Read the model definition and answer for the solid it produces. Units are mm, in the model's axes. Round coordinates to 2 decimals unless told otherwise and drop trailing zeros. Write each loop counter-clockwise with the first axis right and the second up, starting at its lowest first coordinate (ties: lowest second). Pieces come first, ordered by that corner, then holes. Notation, with made-up numbers: (54.25, 65.5) - (68.25, 65.5) arc R28 cw to (68.25, 88.5) - close; hole circle Ø6 at (53, -6). An arc over 180 degrees is marked (long way). One line per item, written item: value. Start each with the question number.
(1) A cutting plane is placed at B-B, the plane x = 0. Determine the outline of the cut face in (y, z), plus the area to 3 significant figures.
(2) The mould has two halves that part along Z. Classify faces 1 (the face through (-39.706, 2.535, -26.086)), 2 (the face through (1, 5, -43)), 3 (the face through (0.811, 2.465, -62.495)): +Z half, -Z half, draft (parallel to the pull), parting line (faces both ways), or undercut.
(3) Find the intervals of material crossed by L1, parallel to X at y = 2.8, z = 25.5; L2, parallel to X at y = 0.35, z = -29.5; L3, parallel to Z at x = 45, y = 4.2, in increasing order.
(4) A cutting plane is placed at A-A, the plane z = 0. Determine the outline of the cut face in (x, y), plus the area to 3 significant figures.
(5) Flat-ended cylindrical pins translate along their axes: pin 1 Ø5.5 at (x, z) = (-44.17, -25.5) entering from +Y; pin 2 Ø3 at (x, y) = (-12.5, 3.5) entering from +Z; pin 3 Ø3 at (x, y) = (26, 4) entering from -Z; pin 4 Ø1 at (y, z) = (3.5, 48.5) entering from +X. Find the tip coordinate at first contact, or state that the pin passes through.
(6) A cutting plane is placed at C-C, the plane z = -25.5. Determine the outline of the cut face in (x, y), plus the area to 3 significant figures.
(7) A cutting plane is placed at D-D, the plane x = -37.5. Determine the outline of the cut face in (y, z), plus the area to 3 significant figures.
from build123d import *

# Parameters (mm, degrees)
SKETCH1_R           = 62.5
SKETCH1_R_2         = 42.5
BOSS_EXTRUDE1_DEPTH = 5
SKETCH2_R           = 4.5
CUT_EXTRUDE1_DEPTH  = 10
SKETCH3_OUTSIDE_W   = 162.37
SKETCH3_OUTSIDE_H   = 162.37
SKETCH3_OUTSIDE_W_2 = 100
SKETCH3_OUTSIDE_H_2 = 143.531180288
CUT_EXTRUDE2_DEPTH  = 10


with BuildPart() as part:
    # Sketch1 → Boss-Extrude1 (new body)
    with BuildSketch(Plane(origin=(0, 0, 0), x_dir=(1, 0, 0), z_dir=(0, 1, 0))):
        with Locations(Location((0, 0, 0), (0, 0, 270))):
            Circle(SKETCH1_R)
        with Locations(Location((0, 0, 0), (0, 0, 270))):
            Circle(SKETCH1_R_2, mode=Mode.SUBTRACT)
    extrude(amount=BOSS_EXTRUDE1_DEPTH)

    # Sketch2 → Cut-Extrude1 (cut)
    with BuildSketch(Plane(origin=(0, 5, 0), x_dir=(1, 0, 0), z_dir=(0, 1, 0))):
        with Locations(Location((0, 51, 0), (0, 0, 270))):
            Circle(SKETCH2_R)
        with Locations(Location((44.167295593, 25.5, 0), (0, 0, 270))):
            Circle(SKETCH2_R)
        with Locations(Location((44.167295593, -25.5, 0), (0, 0, 270))):
            Circle(SKETCH2_R)
        with Locations(Location((0, -51, 0), (0, 0, 270))):
            Circle(SKETCH2_R)
        with Locations(Location((-44.167295593, -25.5, 0), (0, 0, 270))):
            Circle(SKETCH2_R)
        with Locations(Location((-44.167295593, 25.5, 0), (0, 0, 270))):
            Circle(SKETCH2_R)
    extrude(amount=-CUT_EXTRUDE1_DEPTH, mode=Mode.SUBTRACT)

    # Sketch3 outside → Cut-Extrude2 (cut)
    with BuildSketch(Plane(origin=(0, 5, 0), x_dir=(1, 0, 0), z_dir=(0, 1, 0))):
        Rectangle(SKETCH3_OUTSIDE_W, SKETCH3_OUTSIDE_H)
        Rectangle(SKETCH3_OUTSIDE_W_2, SKETCH3_OUTSIDE_H_2, mode=Mode.SUBTRACT)
    extrude(amount=-CUT_EXTRUDE2_DEPTH, mode=Mode.SUBTRACT)


solid = part.part
Here are the results:
1. outline: (0, -62.5) - (5, -62.5) - (5, -55.5) - (0, -55.5) - close; (0, -46.5) - (5, -46.5) - (5, -42.5) - (0, -42.5) - close; (0, 42.5) - (5, 42.5) - (5, 46.5) - (0, 46.5) - close; (0, 55.5) - (5, 55.5) - (5, 62.5) - (0, 62.5) - close
1. area: 110 mm²
2. face 1: undercut
2. face 2: draft
2. face 3: -Z half
3. L1: -50 to -48.67, -39.67 to -34, 34 to 39.67, 48.67 to 50
3. L2: -50 to -46.23, -42.11 to -30.59, 30.59 to 42.11, 46.23 to 50
3. L3: -43.37 to -29.92, -21.08 to 21.08, 29.92 to 43.37
4. outline: (-50, 0) - (-42.5, 0) - (-42.5, 5) - (-50, 5) - close; (42.5, 0) - (50, 0) - (50, 5) - (42.5, 5) - close
4. area: 75.0 mm²
5. pin 1: through
5. pin 2: z = 61.52
5. pin 3: z = -57.5
5. pin 4: x = 40.03
6. outline: (-50, 0) - (-48.67, 0) - (-48.67, 5) - (-50, 5) - close; (-39.67, 0) - (-34, 0) - (-34, 5) - (-39.67, 5) - close; (34, 0) - (39.67, 0) - (39.67, 5) - (34, 5) - close; (48.67, 0) - (50, 0) - (50, 5) - (48.67, 5) - close
6. area: 70.0 mm²
7. outline: (0, -50) - (5, -50) - (5, -20) - (0, -20) - close; (0, 20) - (5, 20) - (5, 50) - (0, 50) - close
7. area: 300 mm²
